Geometry: final body of the model. Coordinates: model frame, mm. A direction names the side the tool comes from. Give positions to 0.01 mm unless a question says otherwise; leave off trailing zeros. Order: outer loops, then holes, each group sorted by start corner. A loop starts at its lowest first (then second) coordinate and runs counter-clockwise, first axis right, second up. Notation, with made-up numbers: (0.5, -25) - (29.5, -25) arc R16 ccw to (29.5, -8) - close; hole circle Ø3 at (-31.5, 67). An arc over 180 degrees is marked (long way). Use one line per item in the form item = value.
from build123d import *

# Parameters (mm, degrees)
SKETCH1_W            = 16.7
SKETCH1_H            = 40
BOSS_EXTRUDE1_DEPTH  = 2
SKETCH12_W           = 16.7
SKETCH12_H           = 40
BOSS_EXTRUDE4_DEPTH  = 6
SKETCH15_R           = 1.5
CUT_EXTRUDE3_DEPTH   = 24.102434937
SKETCH16_W           = 16.7
SKETCH16_H           = 13.250623967
BOSS_EXTRUDE5_DEPTH  = 6
SKETCH21_W           = 16.7
SKETCH21_H           = 13.250623967
BOSS_EXTRUDE10_DEPTH = 4.06
SKETCH22_W           = 16.7
SKETCH22_H           = 4
BOSS_EXTRUDE11_DEPTH = 20
BOSS_EXTRUDE12_DEPTH = 16.7
SKETCH24_R           = 1.5
CUT_EXTRUDE5_DEPTH   = 54.131010889
SKETCH25_W           = 16.7
SKETCH25_H           = 8
BOSS_EXTRUDE13_DEPTH = 2
FILLET1_R            = 2
FILLET2_R            = 2
SKETCH27_W           = 16.7
SKETCH27_H           = 10.06
BOSS_EXTRUDE14_DEPTH = 3
SKETCH26_R           = 1.5
CUT_EXTRUDE6_DEPTH   = 53.215173256
CUT_EXTRUDE7_DEPTH   = 1
FILLET3_R            = 1


with BuildPart() as part:
    # Sketch1 → Boss-Extrude1 (new body)
    with BuildSketch(Plane.XY):
        Rectangle(SKETCH1_W, SKETCH1_H)
    extrude(amount=BOSS_EXTRUDE1_DEPTH)

    # Sketch12 → Boss-Extrude4 (add)
    with BuildSketch(Plane(origin=(0, 0, 0), x_dir=(-1, 0, 0), z_dir=(0, 0, -1))):
        Rectangle(SKETCH12_W, SKETCH12_H)
    extrude(amount=BOSS_EXTRUDE4_DEPTH)

    # Sketch15 → Cut-Extrude3 (cut, through all)
    with BuildSketch(Plane.XY.offset(2)):
        with Locations((0, 12.5)):
            Circle(SKETCH15_R)
        with Locations((0, -12.5)):
            Circle(SKETCH15_R)
    extrude(amount=-CUT_EXTRUDE3_DEPTH, mode=Mode.SUBTRACT)

    # Sketch16 → Boss-Extrude5 (add)
    with BuildSketch(Plane(origin=(0, 0, -6), x_dir=(-1, 0, 0), z_dir=(0, 0, -1))):
        with Locations((0, 23.926623866)):
            Rectangle(SKETCH16_W, SKETCH16_H)
        with Locations((0, -23.926623866)):
            Rectangle(SKETCH16_W, SKETCH16_H)
    extrude(amount=BOSS_EXTRUDE5_DEPTH)

    # Sketch21 → Boss-Extrude10 (add)
    with BuildSketch(Plane(origin=(0, 0, -12), x_dir=(-1, 0, 0), z_dir=(0, 0, -1))):
        with Locations((0, -23.926623866)):
            Rectangle(SKETCH21_W, SKETCH21_H)
        with Locations((0, 23.926623866)):
            Rectangle(SKETCH21_W, SKETCH21_H)
    extrude(amount=BOSS_EXTRUDE10_DEPTH)

    # Sketch22 → Boss-Extrude11 (add)
    with BuildSketch(Plane.XZ.offset(30.551935849)):
        with Locations((0, -14.06)):
            Rectangle(SKETCH22_W, SKETCH22_H)
    extrude(amount=BOSS_EXTRUDE11_DEPTH)

    # Sketch23 → Boss-Extrude12 (add)
    with BuildSketch(Plane(origin=(8.35, 0, 0), x_dir=(0, 0, -1), z_dir=(1, 0, 0))):
        Polygon((-2, -20), (6, -30.551935849), (12.06, -38.545027255), (12.06, -20), align=None)
    extrude(amount=-BOSS_EXTRUDE12_DEPTH)

    # Sketch24 → Cut-Extrude5 (cut, through all)
    with BuildSketch(Plane.XY.offset(-12.06)):
        with Locations((0, -44.548481552)):
            Circle(SKETCH24_R)
        with Locations((0, 44.548481552)):
            Circle(SKETCH24_R)
    extrude(amount=-CUT_EXTRUDE5_DEPTH, mode=Mode.SUBTRACT)

    # Sketch25 → Boss-Extrude13 (add)
    with BuildSketch(Plane(origin=(0, 20, 0), x_dir=(1, 0, 0), z_dir=(0, 1, 0))):
        with Locations((0, 2)):
            Rectangle(SKETCH25_W, SKETCH25_H)
    extrude(amount=BOSS_EXTRUDE13_DEPTH)

    # Fillet1
    fillet1_edges = [part.edges().sort_by_distance(p)[0] for p in [
        (0, 22, 2),
    ]]
    fillet(fillet1_edges, radius=FILLET1_R)

    # Fillet2
    fillet2_edges = [part.edges().sort_by_distance(p)[0] for p in [
        (0, 22, -6),
    ]]
    fillet(fillet2_edges, radius=FILLET2_R)

    # Sketch27 → Boss-Extrude14 (add)
    with BuildSketch(Plane(origin=(0, 30.551935849, 0), x_dir=(1, 0, 0), z_dir=(0, 1, 0))):
        with Locations((0, 11.03)):
            Rectangle(SKETCH27_W, SKETCH27_H)
    extrude(amount=BOSS_EXTRUDE14_DEPTH)

    # Sketch26 → Cut-Extrude6 (cut, through all)
    with BuildSketch(Plane.XY.offset(-6)):
        with Locations((0, 28.951518448)):
            Circle(SKETCH26_R)
    extrude(amount=-CUT_EXTRUDE6_DEPTH, mode=Mode.SUBTRACT)

    # Sketch28 → Cut-Extrude7 (cut)
    with BuildSketch(Plane.ZY.offset(8.35)):
        with BuildLine():
            Line((2, -20), (2, 20))
            ThreePointArc((2, 20), (1.414213562, 21.414213562), (0, 22))
            Line((0, 22), (-4, 22))
            ThreePointArc((-4, 22), (-5.414213562, 22.585786438), (-6, 24))
            Line((-6, 24), (-6, 33.551935849))
            Line((-6, 33.551935849), (-16.06, 33.551935849))
            Line((-16.06, 33.551935849), (-16.06, 17.301311882))
            Line((-16.06, 17.301311882), (-6, 17.301311882))
            Line((-6, 17.301311882), (-6, -17.301311882))
            Line((-6, -17.301311882), (-16.06, -17.301311882))
            Line((-16.06, -17.301311882), (-16.06, -50.551935849))
            Line((-16.06, -50.551935849), (-12.06, -50.551935849))
            Line((-12.06, -50.551935849), (-12.06, -38.545027255))
            Line((-12.06, -38.545027255), (2, -20))
        make_face()
    extrude(amount=-CUT_EXTRUDE7_DEPTH, mode=Mode.SUBTRACT)

    # Fillet3
    fillet3_edges = [part.edges().sort_by_distance(p)[0] for p in [
        (0.5, 33.551935849, -6),
        (0.5, -20, 2),
        (0.5, -38.545027255, -12.06),
        (0.5, -17.301311882, -6),
        (0.5, 17.301311882, -6),
        (0.5, -50.551935849, -12.06),
    ]]
    fillet(fillet3_edges, radius=FILLET3_R)


solid = part.part
(1) Cut plane C-C on x = 5. Output: boundary loops of the cut face in (y, z).
Computed values:
outline = (-50.55, -16.06) - (-17.3, -16.06) - (-17.3, -7) arc R1 cw to (-16.3, -6) - (16.3, -6) arc R1 cw to (17.3, -7) - (17.3, -16.06) - (33.55, -16.06) - (33.55, -7) arc R1 ccw to (32.55, -6) - (24, -6) arc R2 cw to (22, -4) - (22, 0) arc R2 ccw to (20, 2) - (-19.66, 2) arc R1 ccw to (-20.27, 1.8) - (-38.28, -11.86) arc R1 cw to (-38.88, -12.06) - (-49.55, -12.06) arc R1 ccw to (-50.55, -13.06) - close
(2) Pull-direction query (Y, two-part tool) for faces 1 (the face through (1, -17.301, -11)), 2 (the face through (0.61, 21.4, 1.43)), 3 (the face through (2, -44, -12.06)); classes: released by +Y, released by -Y, zero draft, split by the parting line, or undercut.
Computed values:
face_1 = undercut
face_2 = released by +Y
face_3 = zero draft
(3) Ray query, line 1 along Y through (x, z) = (0, -13.2); line 2 along Y through (x, z) = (1.75, -13.25); line 3 along Z through (x, y) = (-2, -3.5). Return the intervals inside material, ascending.
Computed values:
line_1 = -50.55 to -46.05, -43.05 to -17.3, 17.3 to 27.45, 30.45 to 33.55
line_2 = -50.55 to -17.3, 17.3 to 33.55
line_3 = -6 to 2
(4) Cut plane A-A on y = -12.5. Output: boundary loops of the cut face in (x, z).
Computed values:
outline = (-7.35, -6) - (-1.5, -6) - (-1.5, 2) - (-7.35, 2) - close; (1.5, -6) - (8.35, -6) - (8.35, 2) - (1.5, 2) - close
(5) Contact query for flat-ended pins moving along their axis: pin 1 Ø5 at (y, z) = (-39.5, -8.5) entering from +X; pin 2 Ø10 at (y, z) = (-41, -10.5) entering from +X; pin 3 Ø8.5 at (x, y) = (3, -45) entering from +Z; pin 4 Ø4 at (x, y) = (0, -12.5) entering from -Z. Output: stop coordinate, or through.
Computed values:
pin_1 = through
pin_2 = 8.35
pin_3 = -12.06
pin_4 = -6
(6) Reachability of faces 4 (the face through (1, 17.301, -11)), 5 (the face through (0, 27, -6)), 6 (the face through (0, -50.552, -15)) from +Z, -Z, +X, -X, +Y, -Y: full face, straight path, thin tool, end or side. Return the list, or none.
Computed values:
face_4 = -Z, +X, -X
face_5 = +Z, +X, -X, +Y
face_6 = +Z, -Z, +X, -X, -Y
(7) Cut plane B-B on z = -14. Output: boundary loops of the cut face in (x, y), plus the area to 3 significant figures.
Computed values:
outline = (-7.35, -50.55) - (8.35, -50.55) - (8.35, -17.3) - (-7.35, -17.3) - close; (-7.35, 17.3) - (8.35, 17.3) - (8.35, 33.55) - (-7.35, 33.55) - close; hole circle Ø3 at (0, -44.55); hole circle Ø3 at (0, 28.95)
area = 763 mm²
(8) Cut plane D-D on z = -1.75. Output: boundary loops of the cut face in (x, y), plus the area to 3 significant figures.
Computed values:
outline = (-7.35, -24.95) - (8.35, -24.95) - (8.35, 22) - (-7.35, 22) - close; hole circle Ø3 at (0, -12.5); hole circle Ø3 at (0, 12.5)
area = 723 mm²
